The model under review builds one solid part; all positions refer to its coordinate system, in mm. A direction names the side the tool comes from. Coordinates: 2 decimals unless noted, no trailing zeros. Write each loop counter-clockwise with the first axis right and the second up, starting at its lowest first coordinate (ties: lowest second). Pieces come first, ordered by that corner, then holes. Notation, with made-up numbers: (41.5, -4.5) -> (71.5, -4.5) arc R33 ccw to (71.5, 24.5) -> close; hole circle Ø11 at (45.5, 88). An arc over 180 degrees is marked (long way). Write each question's results on one line, items separated by ' | '.
```python
from build123d import *

# Parameters (mm, degrees)
SKETCH1_R           = 10
BOSS_EXTRUDE1_DEPTH = 10
SKETCH2_R           = 16
BOSS_EXTRUDE2_DEPTH = 5
CHAMFER1_SIZE       = 1
SKETCH3_R           = 2
CUT_EXTRUDE1_DEPTH  = 10
CIRPATTERN1_COUNT   = 4
SKETCH4_R           = 5.5
CUT_EXTRUDE2_DEPTH  = 29


with BuildPart() as part:
    # Sketch1 → Boss-Extrude1 (new body)
    with BuildSketch(Plane.XY):
        Circle(SKETCH1_R)
    extrude(amount=BOSS_EXTRUDE1_DEPTH)

    # Sketch2 → Boss-Extrude2 (add)
    with BuildSketch(Plane.XY.offset(10)):
        Circle(SKETCH2_R)
    extrude(amount=BOSS_EXTRUDE2_DEPTH)

    # Chamfer1
    chamfer1_edges = [part.edges().sort_by_distance(p)[0] for p in [
        (-10, 0, 0),
        (-16, 0, 15),
    ]]
    chamfer(chamfer1_edges, length=CHAMFER1_SIZE)

    # Sketch3 → Cut-Extrude1 (cut)
    with BuildSketch(Plane(origin=(0, 0, 10), x_dir=(-1, 0, 0), z_dir=(0, 0, -1))):
        with Locations((0, 13)):
            Circle(SKETCH3_R)
    cut_extrude1 = extrude(amount=-CUT_EXTRUDE1_DEPTH, mode=Mode.SUBTRACT)

    # CirPattern1: Cut-Extrude1 ×4 about axis
    cirpattern1_axis = Axis((0, 0, 0), (0, 0, 1))
    for i in range(1, CIRPATTERN1_COUNT):
        add(cut_extrude1.rotate(cirpattern1_axis, i * 360 / CIRPATTERN1_COUNT), mode=Mode.SUBTRACT)

    # Sketch4 → Cut-Extrude2 (cut)
    with BuildSketch(Plane(origin=(0, 0, 0), x_dir=(-1, 0, 0), z_dir=(0, 0, -1))):
        Circle(SKETCH4_R)
    extrude(amount=-CUT_EXTRUDE2_DEPTH, mode=Mode.SUBTRACT)


solid = part.part
```
Q1. Clearance check with flat-ended pins moving along their axes: P1, Ø4, axis at y = -6, z = 7, coming from the +X side; P2, Ø2, axis at y = -9, z = 1.5, coming from the -X side; P3, Ø4.5, axis at x = 0, y = -13, coming from the -Z side; P4, Ø12.5, axis at x = 0, y = 0, coming from the -Z side. State where each tip first meets the part, or that it passes through.
Solution:
P1: x = 9.17 | P2: x = -6 | P3: z = 10 | P4: z = 0
Q2. Machinability: for faces 1 (the cylindrical face through (-2.17, -9.76, 5.44)), 2 (the cylindrical face through (0, 15, 12)), which of the approach directions +Z, -Z, +X, -X, +Y, -Y give a long, thin tool a straight path to every point of the face, cutting with its end or side? Answer none if there is none.
Solution:
face 1: -Z | face 2: +Z, -Z
Q3. Add section B-B (z = 3). Write out the cut boundary in (x, y).
Solution:
outline: circle Ø20 at (0, 0); hole circle Ø11 at (0, 0)
Q4. For line 1 (Y direction, x = 0, z = 12.6); line 2 (X direction, y = 0.5, z = 13.75); line 3 (Y direction, x = -3, z = 8.5), list the stretches that pass through material, from the lowest coordinate up. Write a range as from..to.
Solution:
line 1: -16..-15, -11..-5.5, 5.5..11, 15..16 | line 2: -15.99..-14.94, -11.06..-5.48, 5.48..11.06, 14.94..15.99 | line 3: -9.54..-4.61, 4.61..9.54
Q5. Add section A-A (z = 12). Write out the cut boundary in (x, y).
Solution:
outline: circle Ø32 at (0, 0); hole circle Ø4 at (-13, 0); hole circle Ø11 at (0, 0); hole circle Ø4 at (0, -13); hole circle Ø4 at (0, 13); hole circle Ø4 at (13, 0)
